from build123d import *

# Parameters (mm, degrees)
SKETCH1_W                      = 200
SKETCH1_H                      = 500
BOSS_EXTRUDE1_DEPTH            = 12
SKETCH2_R                      = 20
SKETCH2_R_2                    = 11
CUT_EXTRUDE1_DEPTH             = 12
SKETCH4_R                      = 12.5
CUT_EXTRUDE3_DEPTH             = 12
SKETCH5_R                      = 7
CUT_EXTRUDE4_DEPTH             = 12
F_8_2_8_2_DIAMETER_HOLE1_D     = 8.2
F_8_2_8_2_DIAMETER_HOLE1_DEPTH = 13
F_8_2_8_2_DIAMETER_HOLE1_TIP   = 2.463528538
F_10_0_10_DIAMETER_HOLE1_D     = 10
SKETCH11_W                     = 47
SKETCH11_H                     = 47
CUT_EXTRUDE6_DEPTH             = 270.525508997
CUT_EXTRUDE7_DEPTH             = 270.525508997
F_5_0_5_DIAMETER_HOLE1_D       = 5
CUT_EXTRUDE8_DEPTH             = 270.525508997


with BuildPart() as part:
    # Sketch1 → Boss-Extrude1 (new body)
    with BuildSketch(Plane(origin=(0, 0, 0), x_dir=(1, 0, 0), z_dir=(0, 1, 0))):
        Rectangle(SKETCH1_W, SKETCH1_H)
    extrude(amount=BOSS_EXTRUDE1_DEPTH)

    # Sketch2 → Cut-Extrude1 (cut)
    with BuildSketch(Plane(origin=(0, 12, 0), x_dir=(1, 0, 0), z_dir=(0, 1, 0))):
        with Locations(Location((-50, 0, 0), (0, 0, 270))):
            Circle(SKETCH2_R)
        with Locations(Location((-50, 120, 0), (0, 0, 270))):
            Circle(SKETCH2_R_2)
        with Locations(Location((-50, -120, 0), (0, 0, 90))):
            Circle(SKETCH2_R_2)
    extrude(amount=-CUT_EXTRUDE1_DEPTH, mode=Mode.SUBTRACT)

    # Sketch4 → Cut-Extrude3 (cut)
    with BuildSketch(Plane(origin=(0, 12, 0), x_dir=(1, 0, 0), z_dir=(0, 1, 0))):
        with Locations(Location((40, 180, 0), (0, 0, 270))):
            Circle(SKETCH4_R)
        with Locations(Location((40, -180, 0), (0, 0, 90))):
            Circle(SKETCH4_R)
    extrude(amount=-CUT_EXTRUDE3_DEPTH, mode=Mode.SUBTRACT)

    # Sketch5 → Cut-Extrude4 (cut)
    with BuildSketch(Plane(origin=(0, 12, 0), x_dir=(1, 0, 0), z_dir=(0, 1, 0))):
        with Locations(Location((-77.5, 227.5, 0), (0, 0, 270))):
            Circle(SKETCH5_R)
        with Locations(Location((77.5, 227.5, 0), (0, 0, 270))):
            Circle(SKETCH5_R)
        with Locations(Location((-77.5, -227.5, 0), (0, 0, 270))):
            Circle(SKETCH5_R)
        with Locations(Location((77.5, -227.5, 0), (0, 0, 270))):
            Circle(SKETCH5_R)
    extrude(amount=-CUT_EXTRUDE4_DEPTH, mode=Mode.SUBTRACT)

    # Ø8.2 (8.2) Diameter Hole1
    with Locations(Plane(origin=(0, 12, 0), x_dir=(1, 0, 0), z_dir=(0, 1, 0))):
        with Locations((85, 177.098099642), (85, 70), (85, -70), (85, -150)):
            Hole(F_8_2_8_2_DIAMETER_HOLE1_D / 2, depth=F_8_2_8_2_DIAMETER_HOLE1_DEPTH)
            with Locations((0, 0, -(F_8_2_8_2_DIAMETER_HOLE1_DEPTH + F_8_2_8_2_DIAMETER_HOLE1_TIP / 2))):  # 118° drill point
                Cone(0, F_8_2_8_2_DIAMETER_HOLE1_D / 2, F_8_2_8_2_DIAMETER_HOLE1_TIP, mode=Mode.SUBTRACT)

    # Ø10.0 (10) Diameter Hole1 (through all)
    with Locations(Plane(origin=(0, 12, 0), x_dir=(1, 0, 0), z_dir=(0, 1, 0))):
        with Locations((-30, 227.5), (30, 227.5), (30, -227.5), (-30, -227.5)):
            Hole(F_10_0_10_DIAMETER_HOLE1_D / 2)

    # Sketch11 → Cut-Extrude6 (cut, through all)
    with BuildSketch(Plane(origin=(0, 12, 0), x_dir=(1, 0, 0), z_dir=(0, 1, 0))):
        with Locations((-76.5, 226.5)):
            Rectangle(SKETCH11_W, SKETCH11_H)
        with Locations((-76.5, -226.5)):
            Rectangle(SKETCH11_W, SKETCH11_H)
    extrude(amount=-CUT_EXTRUDE6_DEPTH, mode=Mode.SUBTRACT)

    # Sketch3 → Cut-Extrude7 (cut, through all)
    with BuildSketch(Plane(origin=(0, 12, 0), x_dir=(1, 0, 0), z_dir=(0, 1, 0))):
        with BuildLine():
            Line((50, -37.5), (40, -37.5))
            ThreePointArc((40, -37.5), (2.5, 0), (40, 37.5))
            Line((40, 37.5), (50, 37.5))
            ThreePointArc((50, 37.5), (87.5, 0), (50, -37.5))
        make_face()
    extrude(amount=-CUT_EXTRUDE7_DEPTH, mode=Mode.SUBTRACT)

    # Ø5.0 (5) Diameter Hole1 (through all)
    with Locations(Plane(origin=(0, 12, 0), x_dir=(1, 0, 0), z_dir=(0, 1, 0))):
        with Locations((5.15, 34.85), (5.15, -34.85), (74.85, -34.85), (74.85, 34.85)):
            Hole(F_5_0_5_DIAMETER_HOLE1_D / 2)

    # Sketch16 → Cut-Extrude8 (cut, through all)
    with BuildSketch(Plane(origin=(0, 12, 0), x_dir=(1, 0, 0), z_dir=(0, 1, 0))):
        with BuildLine():
            Line((5.15, 38.15), (15.15, 38.15))
            ThreePointArc((15.15, 38.15), (18.45, 34.85), (15.15, 31.55))
            Line((15.15, 31.55), (5.15, 31.55))
            ThreePointArc((5.15, 31.55), (1.85, 34.85), (5.15, 38.15))
        make_face()
        with BuildLine():
            Line((74.85, 38.15), (84.85, 38.15))
            ThreePointArc((84.85, 38.15), (88.15, 34.85), (84.85, 31.55))
            Line((84.85, 31.55), (74.85, 31.55))
            ThreePointArc((74.85, 31.55), (71.55, 34.85), (74.85, 38.15))
        make_face()
        with BuildLine():
            Line((5.15, -31.55), (15.15, -31.55))
            ThreePointArc((15.15, -31.55), (18.45, -34.85), (15.15, -38.15))
            Line((15.15, -38.15), (5.15, -38.15))
            ThreePointArc((5.15, -38.15), (1.85, -34.85), (5.15, -31.55))
        make_face()
        with BuildLine():
            Line((74.85, -31.55), (84.85, -31.55))
            ThreePointArc((84.85, -31.55), (88.15, -34.85), (84.85, -38.15))
            Line((84.85, -38.15), (74.85, -38.15))
            ThreePointArc((74.85, -38.15), (71.55, -34.85), (74.85, -31.55))
        make_face()
    extrude(amount=-CUT_EXTRUDE8_DEPTH, mode=Mode.SUBTRACT)


solid = part.part
The model under review builds one solid part; all positions refer to its coordinate system, in mm. A direction names the side the tool comes from. Give positions to 0.01 mm unless a question says otherwise; leave off trailing zeros. Order: outer loops, then holes, each group sorted by start corner. A loop starts at its lowest first (then second) coordinate and runs counter-clockwise, first axis right, second up. Notation, with made-up numbers: M -30.5,-23 L -18.5,-23 A26 cw -18.5,5 Z; hole C 81,53 d5. An arc over 180 degrees is marked long. One line per question, with ' | ' between items. Start each with the question number.
1) Consider section D-D, the plane y = 7.5. State how many separate pieces and enclosed holes the cut face has, then the cut area to 3 significant figures.
2) Clearance check with flat-ended pins moving along their axes: P1, Ø3.5, axis at y = 5.5, z = 220, coming from the -X side; P2, Ø6, axis at x = -70, y = 8.5, coming from the -Z side. State where each tip first meets the part, or that it passes through.
3) Consider section A-A, the plane z = 0. Give the boundary of the cut face in (x, y).
4) Wall thickness on L1, parallel to X at y = 8.5, z = -227.5; L2, parallel to Z at x = 79.5, y = 5.75; L3, parallel to Z at x = 30, y = 8.25: over which ranges is each line inside the solid? List them lowest first. Write a range as from..to.
5) Mouldability with a two-part tool opening along X and no side actions: class faces 1 (the face through (-77, 6, 203)), 2 (the face through (-100, 6, 3)), 3 (the face through (35.212, 6.084, -168.453)) as pulls with the +X half, pulls with the -X half, needs draft (parallel to the pull), parting line crosses it, or undercut.
6) For faces 4 (the face through (80, 6, -38.15)), 5 (the face through (-77, 6, -203)), 6 (the face through (-1, 12, -4)), list the 3-axis set-ups (+Z, -Z, +X, -X, +Y, -Y) from which the entire face can be reached by the end or side of a thin tool; tool diameter is ignored.
7) Consider section C-C, the plane z = -120. Give the boundary of the cut face in (x, y).
8) Consider section B-B, the plane z = -227.5. Give the boundary of the cut face in (x, y).
Found:
1) separate pieces: 1 | enclosed holes: 20 | area: 86,200 mm²
2) P1: stops at x = -53 | P2: stops at z = -203
3) outline: M -100,0 L -70,0 L -70,12 L -100,12 Z; M -30,0 L 2.5,0 L 2.5,12 L -30,12 Z; M 87.5,0 L 100,0 L 100,12 L 87.5,12 Z
4) L1: x = -53..-35, -25..25, 35..70.5, 84.5..100 | L2: z = -250..-234.21, -220.79..-38.15, -31.55..-23.15, 23.15..31.55, 38.15..220.79, 234.21..250 | L3: z = -250..-232.5, -222.5..-187.5, -172.5..-36.14, 36.14..172.5, 187.5..222.5, 232.5..250
5) face 1: needs draft | face 2: pulls with the -X half | face 3: undercut
6) face 4: +Y, -Y | face 5: -Z, -X, +Y, -Y | face 6: +Z, -Z, +X, -X, +Y
7) outline: M -100,0 L -61,0 L -61,12 L -100,12 Z; M -39,0 L 100,0 L 100,12 L -39,12 Z
8) outline: M -53,0 L -35,0 L -35,12 L -53,12 Z; M -25,0 L 25,0 L 25,12 L -25,12 Z; M 35,0 L 70.5,0 L 70.5,12 L 35,12 Z; M 84.5,0 L 100,0 L 100,12 L 84.5,12 Z
